Build history of the part. All positions in model axes, mm. Face numbers are marked on the shaded views. A direction names the side the tool comes from. Round coordinates to 2 decimals unless told otherwise and drop trailing zeros. Write each loop counter-clockwise with the first axis right and the second up, starting at its lowest first coordinate (ties: lowest second). Pieces come first, ordered by that corner, then holes.
Item 1: Wall check: probe 1 along Y at (x, z) = (0.6, 25); probe 2 along Y at (x, z) = (32, 13.5); probe 3 along X at (y, z) = (-40.5, 21). Give the ranges that are in metal, low to high.
Item 2: Mould opens along Y. For the marked faces 1, 2, 3 and 4 say: +Y half, -Y half, draft (parallel to the pull), parting line (faces both ways), or undercut.
Item 3: Band-saw the part on B-B, the plane y = -66. Write the cut outline in (x, z).
Item 4: Drop flat-ended pins along their axis: pin 1 Ø1 at (x, z) = (10.5, 12) entering from +Y; pin 2 Ø2 at (x, z) = (30.5, 7) entering from -Y; pin 3 Ø14.5 at (y, z) = (-59.5, 36.5) entering from +X. Give the stop position or say it passes through.
Item 5: 3-axis set-ups, long thin cutter, end or side, ignore diameter. For the marked faces 5, 6 and 7: which of +Z, -Z, +X, -X, +Y, -Y reach the whole face in a straight line?
Item 6: Band-saw the part on C-C, the plane z = 25. Write the cut outline in (x, y).
Item 7: Band-saw the part on A-A, the plane x = 22. Write the cut outline in (y, z).
Item 8: Band-saw the part on D-D, the plane x = 27.5. Write the cut outline in (y, z).
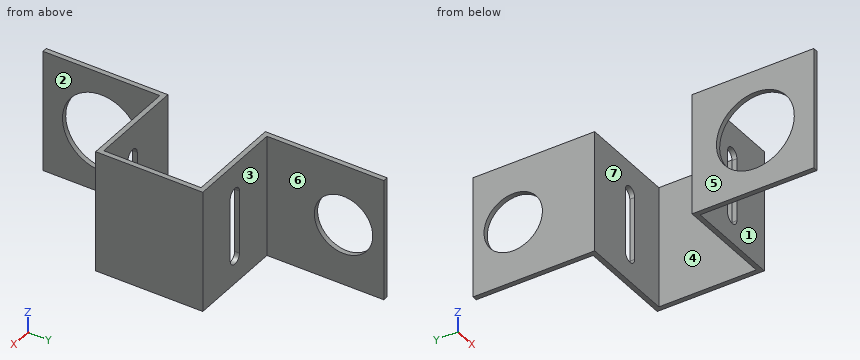
```python
from build123d import *

# Parameters (mm, degrees)
BOSS_EXTRUDE1_DEPTH = 50
CUT_EXTRUDE1_DEPTH  = 50
SKETCH3_R           = 16
CUT_EXTRUDE2_DEPTH  = 50
SKETCH4_R           = 12
CUT_EXTRUDE3_DEPTH  = 50


with BuildPart() as part:
    # Sketch1 → Boss-Extrude1 (new body)
    with BuildSketch(Plane.XY):
        Polygon((0, 50), (0, 0), (40, 0), (40, -40), (0, -40), (0, -90), (2, -90), (2, -42), (42, -42), (42, 2), (2, 2), (2, 50), align=None)
    extrude(amount=BOSS_EXTRUDE1_DEPTH)

    # Sketch2 → Cut-Extrude1 (cut)
    with BuildSketch(Plane(origin=(0, 2, 0), x_dir=(1, 0, 0), z_dir=(0, 1, 0))):
        with BuildLine():
            Line((24.898261367, -11.026648657), (24.898261367, -37.029372299))
            ThreePointArc((24.898261367, -37.029372299), (22, -39.927633667), (19.101738633, -37.029372299))
            Line((19.101738633, -37.029372299), (19.101738633, -11.026648657))
            ThreePointArc((19.101738633, -11.026648657), (22, -8.12838729), (24.898261367, -11.026648657))
        make_face()
    extrude(amount=-CUT_EXTRUDE1_DEPTH, mode=Mode.SUBTRACT)

    # Sketch3 → Cut-Extrude2 (cut)
    with BuildSketch(Plane(origin=(2, 0, 0), x_dir=(0, 0, -1), z_dir=(1, 0, 0))):
        with Locations((-25, -66)):
            Circle(SKETCH3_R)
    extrude(amount=-CUT_EXTRUDE2_DEPTH, mode=Mode.SUBTRACT)

    # Sketch4 → Cut-Extrude3 (cut)
    with BuildSketch(Plane(origin=(2, 0, 0), x_dir=(0, 0, -1), z_dir=(1, 0, 0))):
        with Locations((-25, 33.473514378)):
            Circle(SKETCH4_R)
    extrude(amount=-CUT_EXTRUDE3_DEPTH, mode=Mode.SUBTRACT)


solid = part.part
```
Results:
1. probe 1: y = -90 to -82, -50 to -40, 0 to 21.47, 45.47 to 50
1. probe 2: y = -42 to -40, 0 to 2
1. probe 3: x = 0 to 19.1, 24.9 to 42
2. face 1: -Y half
2. face 2: draft
2. face 3: +Y half
2. face 4: undercut
3. outline: (0, 0) - (2, 0) - (2, 9) - (0, 9) - close; (0, 41) - (2, 41) - (2, 50) - (0, 50) - close
4. pin 1: stops at y = 2
4. pin 2: stops at y = -42
4. pin 3: stops at x = 2
5. face 5: +Z, -Z, -X, +Y, -Y
5. face 6: +Z, -Z, +X, +Y
5. face 7: +Z, -Z, -X
6. outline: (0, -90) - (2, -90) - (2, -82) - (0, -82) - close; (0, -50) - (2, -50) - (2, -42) - (19.1, -42) - (19.1, -40) - (0, -40) - close; (0, 0) - (19.1, 0) - (19.1, 2) - (2, 2) - (2, 21.47) - (0, 21.47) - close; (0, 45.47) - (2, 45.47) - (2, 50) - (0, 50) - close; (24.9, -42) - (42, -42) - (42, 2) - (24.9, 2) - (24.9, 0) - (40, 0) - (40, -40) - (24.9, -40) - close
7. outline: (-42, 0) - (-40, 0) - (-40, 8.13) - (-42, 8.13) - close; (-42, 39.93) - (-40, 39.93) - (-40, 50) - (-42, 50) - close; (0, 0) - (2, 0) - (2, 8.13) - (0, 8.13) - close; (0, 39.93) - (2, 39.93) - (2, 50) - (0, 50) - close
8. outline: (-42, 0) - (-40, 0) - (-40, 50) - (-42, 50) - close; (0, 0) - (2, 0) - (2, 50) - (0, 50) - close
